Verification items for the finished model (mm, model axes). Give positions to 0.01 mm unless a question says otherwise; leave off trailing zeros. Write each loop counter-clockwise with the first axis right and the second up, starting at its lowest first coordinate (ties: lowest second). Pieces come first, ordered by that corner, then holes. Notation, with made-up numbers: (54, -23) -> (105, -23) arc R19 cw to (105, 2) -> close; hole circle Ø5 at (62, 6.25). An arc over 180 degrees is marked (long way). Use one line per item in the form item = value. Start each with the question number.
(1) Section check D-D, the plane y = 83.5. Record the cut outline in (x, z).
(2) Depth check by flat-ended pin: pin 1 Ø15.5 at (x, y) = (0, 90) entering from +Z. Enter the tip coordinate at first touch or a pass-through.
(3) Release check for a two-part mould opening along Y. For faces 1 (the face through (-1, 120, 0)), 2 (the face through (-50, -2, 0)), 3 (the face through (-2.82, -102.69, 0.11)) record: pulls with the +Y half, pulls with the -Y half, needs draft (parallel to the pull), parting line crosses it, or undercut.
(4) Section check C-C, the plane z = 3.75. Record the cut outline in (x, y), plus the area to 3 significant figures.
(5) Section check B-B, the plane x = 0. Record the cut outline in (y, z), plus the area to 3 significant figures.
(6) Section check A-A, the plane y = -90. Record the cut outline in (x, z), plus the area to 3 significant figures.
(7) Scan lines: L1, parallel to Y at x = 0, z = 0; L2, parallel to X at y = 88.5, z = -3.5; L3, parallel to Y at x = -9, z = 5.5. Record each from-to range of solid material in increasing order.
from build123d import *

# Parameters (mm, degrees)
SKETCH1_W           = 100
SKETCH1_H           = 240
BOSS_EXTRUDE1_DEPTH = 7.5
SKETCH2_R           = 13
CUT_EXTRUDE1_DEPTH  = 32


with BuildPart() as part:
    # Sketch1 → Boss-Extrude1 (new, symmetric)
    with BuildSketch(Plane.XY):
        Rectangle(SKETCH1_W, SKETCH1_H)
    extrude(amount=BOSS_EXTRUDE1_DEPTH, both=True)

    # Sketch2 → Cut-Extrude1 (cut)
    with BuildSketch(Plane.XY.offset(7.5)):
        with Locations((0, 90)):
            Circle(SKETCH2_R)
        with Locations((0, -90)):
            Circle(SKETCH2_R)
    extrude(amount=-CUT_EXTRUDE1_DEPTH, mode=Mode.SUBTRACT)


solid = part.part
Completed:
q1.outline = (-50, -7.5) -> (-11.26, -7.5) -> (-11.26, 7.5) -> (-50, 7.5) -> close; (11.26, -7.5) -> (50, -7.5) -> (50, 7.5) -> (11.26, 7.5) -> close
q2.pin_1 = through
q3.face_1 = pulls with the +Y half
q3.face_2 = needs draft
q3.face_3 = undercut
q4.outline = (-50, -120) -> (50, -120) -> (50, 120) -> (-50, 120) -> close; hole circle Ø26 at (0, -90); hole circle Ø26 at (0, 90)
q4.area = 22,900 mm²
q5.outline = (-120, -7.5) -> (-103, -7.5) -> (-103, 7.5) -> (-120, 7.5) -> close; (-77, -7.5) -> (77, -7.5) -> (77, 7.5) -> (-77, 7.5) -> close; (103, -7.5) -> (120, -7.5) -> (120, 7.5) -> (103, 7.5) -> close
q5.area = 2,820 mm²
q6.outline = (-50, -7.5) -> (-13, -7.5) -> (-13, 7.5) -> (-50, 7.5) -> close; (13, -7.5) -> (50, -7.5) -> (50, 7.5) -> (13, 7.5) -> close
q6.area = 1,110 mm²
q7.L1 = -120 to -103, -77 to 77, 103 to 120
q7.L2 = -50 to -12.91, 12.91 to 50
q7.L3 = -120 to -99.38, -80.62 to 80.62, 99.38 to 120
